```python
from build123d import *

# Parameters (mm, degrees)
SKETCH_1_R             = 7.5
EXTRUDE_1_DEPTH        = 6
HOLE_WIZARD_M6_1_D     = 5
HOLE_WIZARD_M6_1_DEPTH = 25
HOLE_WIZARD_M6_1_TIP   = 1.443375673


with BuildPart() as part:
    # 草图1 → 凸台-拉伸1 (new, symmetric)
    with BuildSketch(Plane(origin=(0, 0, -465), x_dir=(-1, 0, 0), z_dir=(0, 0, -1))):
        Polygon((-557.085724054, 1805.000303929), (-557.085724054, 1591.500303929), (-647.085724054, 1591.500303929), (-647.085724054, 1805.000303929), (-697.085724054, 1805.000303929), (-697.085724054, 1505.000303929), (-647.085724054, 1505.000303929), (-647.085724054, 1555.000303929), (-557.085724054, 1555.000303929), (-557.085724054, 1505.000303929), (-507.085724054, 1505.000303929), (-507.085724054, 1805.000303929), align=None)
        with Locations((-553.939078063, 1570.019037425)):
            Circle(SKETCH_1_R, mode=Mode.SUBTRACT)
        with Locations((-645.939078063, 1570.019037425)):
            Circle(SKETCH_1_R, mode=Mode.SUBTRACT)
    extrude(amount=EXTRUDE_1_DEPTH, both=True)

    # M6 螺纹孔1
    with Locations(Plane(origin=(0, 1805.000303929, 0), x_dir=(1, 0, 0), z_dir=(0, 1, 0))):
        with Locations((672.085724054, 465), (532.085724054, 465)):
            Hole(HOLE_WIZARD_M6_1_D / 2, depth=HOLE_WIZARD_M6_1_DEPTH)
            with Locations((0, 0, -(HOLE_WIZARD_M6_1_DEPTH + HOLE_WIZARD_M6_1_TIP / 2))):  # 120° drill point
                Cone(0, HOLE_WIZARD_M6_1_D / 2, HOLE_WIZARD_M6_1_TIP, mode=Mode.SUBTRACT)


solid = part.part
```
The model under review builds one solid part; all positions refer to its coordinate system, in mm. A direction names the side the tool comes from. Round coordinates to 2 decimals unless told otherwise and drop trailing zeros. Loops run counter-clockwise (first coordinate to the right, second up) from the corner with the lowest first, then second, coordinate; pieces in that order, holes last. Notation, with made-up numbers: (44.5, 17) - (100.5, 17) arc R25 cw to (100.5, 44) - close; hole circle Ø1 at (64.5, 74.5). An arc over 180 degrees is marked (long way). Use a Markdown table: item, result. Add a question column.
Q1. Machinability: for faces 4 (the face through (557.086, 1530, -465)), 5 (the face through (603, 1590, -471)), 6 (the face through (647.086, 1697, -465)), which of the approach directions +Z, -Z, +X, -X, +Y, -Y give a long, thin tool a straight path to every point of the face, cutting with its end or side? Answer none if there is none.
Q2. Add section A-A (y = 1649.5). State the section outline as (x, z) points.
Q3. Add section C-C (x = 620.5). State the section outline as (y, z) points.
Q4. Insertion check: pin 1 Ø4.5 at (x, z) = (532.09, -465) entering from +Y; pin 2 Ø6 at (x, z) = (623, -463.5) entering from +Y; pin 3 Ø3 at (x, z) = (672.09, -465) entering from +Y; pin 4 Ø13.5 at (x, y) = (645.94, 1570.02) entering from +Z. Each pin has a flat end and moves straight along its axis. Give the tip position at first contact, or say it passes through.
Q5. For probe 1 along X at (y, z) = (1799, -465); probe 2 along X at (y, z) = (1658, -464.25); probe 3 along Y at (x, z) = (620, -459.75), list the stretches that pass through material, from the lowest coordinate up.
Q6. The part is to be moulded in two halves that separate along Y. For faces 1 (the face through (532, 1805, -468)), 2 (the face through (532, 1505, -465)), 3 (the face through (555.565, 1562.697, -464.916)), say which applies: pulls with the +Y half, pulls with the -Y half, needs draft (parallel to the pull), parting line crosses it, or undercut.
Q7. Add section B-B (y = 1784). State the section outline as (x, z) points.
Worked answers:
| question | item | result |
|---|---|---|
| 1 | face 4 | +Z, -Z, -Y |
| 1 | face 5 | -Z, +X, -X, +Y, -Y |
| 1 | face 6 | +Z, -Z, +Y |
| 2 | outline | (507.09, -471) - (557.09, -471) - (557.09, -459) - (507.09, -459) - close; (647.09, -471) - (697.09, -471) - (697.09, -459) - (647.09, -459) - close |
| 3 | outline | (1555, -471) - (1591.5, -471) - (1591.5, -459) - (1555, -459) - close |
| 4 | pin 1 | y = 1779.86 |
| 4 | pin 2 | y = 1591.5 |
| 4 | pin 3 | y = 1779.43 |
| 4 | pin 4 | through |
| 5 | probe 1 | 507.09 to 529.59, 534.59 to 557.09, 647.09 to 669.59, 674.59 to 697.09 |
| 5 | probe 2 | 507.09 to 557.09, 647.09 to 697.09 |
| 5 | probe 3 | 1555 to 1591.5 |
| 6 | face 1 | pulls with the +Y half |
| 6 | face 2 | pulls with the -Y half |
| 6 | face 3 | undercut |
| 7 | outline | (507.09, -471) - (557.09, -471) - (557.09, -459) - (507.09, -459) - close; (647.09, -471) - (697.09, -471) - (697.09, -459) - (647.09, -459) - close; hole circle Ø5 at (532.09, -465); hole circle Ø5 at (672.09, -465) |
